from build123d import *

# Parameters (mm, degrees)
BOSS_EXTRUDE1_DEPTH = 3
CHAMFER1_SIZE       = 8


with BuildPart() as part:
    # Sketch1 → Boss-Extrude1 (new, symmetric)
    with BuildSketch(Plane.XY):
        Polygon((0, 90), (0, 0), (40, 0), (40, 10), (10, 90), align=None)
    extrude(amount=BOSS_EXTRUDE1_DEPTH, both=True)

    # Chamfer1
    chamfer1_edges = [part.edges().sort_by_distance(p)[0] for p in [
        (0, 0, 0),
    ]]
    chamfer(chamfer1_edges, length=CHAMFER1_SIZE)


solid = part.part
For this review, take the finished solid that the model builds, in its own axes (mm). Give positions to 0.01 mm unless a question says otherwise; leave off trailing zeros. Loops run counter-clockwise (first coordinate to the right, second up) from the corner with the lowest first, then second, coordinate; pieces in that order, holes last. Notation, with made-up numbers: M 41.25,-16.5 L 90.25,-16.5 A14 ccw 90.25,2.5 Z; hole C 30,25 d3. An arc over 180 degrees is marked long. Put each result on its own line as item: value. Start each with the question number.
(1) Add section C-C, the plane x = 3. Write out the cut boundary in (y, z).
(2) Add section A-A, the plane z = -1.5. Write out the cut boundary in (x, y).
(3) Wall thickness on L1, parallel to X at y = 50.5, z = -0.5; L2, parallel to X at y = 82, z = 2.75; L3, parallel to Y at x = 7.5, z = 1.5: over which ranges is each line inside the solid? List them lowest first.
(4) Add section B-B, the plane y = 42. Write out the cut boundary in (x, z).
(5) For pin 1 (1 mm diameter, centred on y = 61, z = 0.5, fed in from +X), flat-tipped, find the tip position at first contact; note if it passes through.
Result:
1. outline: M 5,-3 L 90,-3 L 90,3 L 5,3 Z
2. outline: M 0,8 L 8,0 L 40,0 L 40,10 L 10,90 L 0,90 Z
3. L1: x = 0 to 24.81
3. L2: x = 0 to 13
3. L3: y = 0.5 to 90
4. outline: M 0,-3 L 28,-3 L 28,3 L 0,3 Z
5. pin 1: stops at x = 21.06
